```python
from build123d import *

# Parameters (mm, degrees)
BOSS_EXTRUDE1_DEPTH = 80
SHELL1_T            = -10
SKETCH2_R           = 80
CUT_EXTRUDE1_DEPTH  = 80


with BuildPart() as part:
    # Sketch1 → Boss-Extrude1 (new body)
    with BuildSketch(Plane.XY):
        Polygon((-467.102450828, -35), (-544.884196758, 42.781745931), (-654.884196758, 42.781745931), (-732.665942689, -35), (-732.665942689, -145), (-654.884196758, -222.781745931), (-544.884196758, -222.781745931), (-467.102450828, -145), align=None)
    extrude(amount=BOSS_EXTRUDE1_DEPTH)

    # Shell1
    shell1_openings = [part.faces().sort_by_distance(p)[0] for p in [
        (-599.884196758, -90, 0),
    ]]
    offset(amount=SHELL1_T, openings=shell1_openings, kind=Kind.INTERSECTION)

    # Sketch2 → Cut-Extrude1 (cut)
    with BuildSketch(Plane.XY.offset(80)):
        with Locations((-599.884196758, -90)):
            Circle(SKETCH2_R)
    extrude(amount=-CUT_EXTRUDE1_DEPTH, mode=Mode.SUBTRACT)


solid = part.part
```
Read the model definition and answer for the solid it produces. Units are mm, in the model's axes. A direction names the side the tool comes from. Give positions to 0.01 mm unless a question says otherwise; leave off trailing zeros. Loops run counter-clockwise (first coordinate to the right, second up) from the corner with the lowest first, then second, coordinate; pieces in that order, holes last.
Item 1: Each of these flat-tipped pins is pushed along its axis until it touches: pin 1 Ø5 at (x, z) = (-673.5, 52.5) entering from -Y; pin 2 Ø10 at (x, z) = (-494, 49) entering from -Y; pin 3 Ø8 at (x, z) = (-680, 58) entering from +Y. Where does it stop, or does it pass through?
Item 2: Find the intervals of material crossed by line 1 along Y through (x, z) = (-571, 5); line 2 along X through (y, z) = (-126, 65); line 3 along Z through (x, y) = (-641, 0.5), in increasing order.
Item 3: The mould has two halves that part along Y. Classify faces 3 (the flat face through (-687.207, -176.316, 34.51)), 4 (the flat face through (-505.4, 3.3, 39.4)), 5 (the flat face through (-694.32, -183.346, 39.44)), 6 (the flat face through (-543, -147, 80)): released by +Y, released by -Y, zero draft, split by the parting line, or undercut.
Item 4: The part is cut by section A-A (y = -90). Write down the section's boundary in (x, z), and give its area (3 significant figures).
Item 5: For faces 1 (the flat face through (-512.561, -3.684, 34.51)), 2 (the flat face through (-506.5, -184.4, 39.4)), determine the directions among +Z, -Z, +X, -X, +Y, -Y from which every point of the face is accessible in a straight line to the end or side of a thin tool.
Item 6: The part is cut by section D-D (y = -191). Write down the section's boundary in (x, z).
Item 7: The part is cut by section C-C (x = -540.5). Write down the section's boundary in (y, z).
Item 8: The part is cut by section B-B (z = 21.5). Write down the section's boundary in (x, y), and give its area (3 significant figures).
Taken from the geometry:
1. pin 1: stops at y = -206.67
1. pin 2: stops at y = -176.9
1. pin 3: stops at y = 21.67
2. line 1: y = -222.78 to -212.78, 32.78 to 42.78
2. line 2: x = -732.67 to -722.67, -477.1 to -467.1
2. line 3: z = 70 to 80
3. face 3: undercut
3. face 4: released by +Y
3. face 5: released by -Y
3. face 6: zero draft
4. outline: (-732.67, 0) - (-722.67, 0) - (-722.67, 70) - (-679.88, 70) - (-679.88, 80) - (-732.67, 80) - close; (-519.88, 70) - (-477.1, 70) - (-477.1, 0) - (-467.1, 0) - (-467.1, 80) - (-519.88, 80) - close
4. area: 2,460 mm2
5. face 1: -Z
5. face 2: +Z, -Z, +X, -Y
6. outline: (-686.67, 0) - (-672.52, 0) - (-672.52, 70) - (-527.24, 70) - (-527.24, 0) - (-513.1, 0) - (-513.1, 80) - (-686.67, 80) - close
7. outline: (-218.4, 0) - (-204.26, 0) - (-204.26, 70) - (-143.61, 70) - (-143.61, 80) - (-218.4, 80) - close; (-36.39, 70) - (24.26, 70) - (24.26, 0) - (38.4, 0) - (38.4, 80) - (-36.39, 80) - close
8. outline: (-732.67, -145) - (-654.88, -222.78) - (-544.88, -222.78) - (-467.1, -145) - (-467.1, -35) - (-544.88, 42.78) - (-654.88, 42.78) - (-732.67, -35) - close; hole (-722.67, -140.86) - (-650.74, -212.78) - (-549.03, -212.78) - (-477.1, -140.86) - (-477.1, -39.14) - (-549.03, 32.78) - (-650.74, 32.78) - (-722.67, -39.14) - close
8. area: 8,470 mm2
